```python
from build123d import *

# Parameters (mm, degrees)
JAW_BODY_DEPTH         = 64
PIVOT_BOSS_DEPTH       = 22
PIVOT_BORE_SKETCH_R    = 6
PIVOT_BORE_12_DEPTH    = 32
GUIDE_KEY_SKETCH_W     = 16
GUIDE_KEY_SKETCH_H     = 9
GUIDE_KEY_DEPTH        = 32
PIVOT_BOSS_FILLET_R3_R = 3
COUNTERBORE_SKETCH_R   = 5
COUNTERBORE_10X4_DEPTH = 4
SCREW_HOLE_SKETCH_R    = 3
SCREW_HOLE_6X4_DEPTH   = 4


with BuildPart() as part:
    # Jaw Body Profile Sketch → Jaw Body (new body)
    with BuildSketch(Plane.XY):
        Polygon((0, 0), (32, 0), (32, 10), (10, 10), (10, 36), (0, 36), align=None)
    extrude(amount=-JAW_BODY_DEPTH)

    # Pivot Boss Sketch → Pivot Boss (add)
    with BuildSketch(Plane(origin=(32, 0, 0), x_dir=(0, 0, -1), z_dir=(1, 0, 0))):
        with BuildLine():
            Line((4.5, 10), (16.574185034, 28.68413566))
            ThreePointArc((16.574185034, 28.68413566), (28.969550727, 35.965977968), (42.206819819, 30.358391585))
            Line((42.206819819, 30.358391585), (59.5, 10))
            Line((59.5, 10), (4.5, 10))
        make_face()
    extrude(amount=-PIVOT_BOSS_DEPTH)

    # Pivot Bore Sketch → Pivot Bore Ø12 (cut)
    with BuildSketch(Plane(origin=(32, 0, 0), x_dir=(0, 0, -1), z_dir=(1, 0, 0))):
        with Locations((30.01240619, 20)):
            Circle(PIVOT_BORE_SKETCH_R)
    extrude(amount=-PIVOT_BORE_12_DEPTH, mode=Mode.SUBTRACT)

    # Guide Key Sketch → Guide Key (add)
    with BuildSketch(Plane(origin=(32, 0, 0), x_dir=(0, 0, -1), z_dir=(1, 0, 0))):
        with Locations((32, -4.5)):
            Rectangle(GUIDE_KEY_SKETCH_W, GUIDE_KEY_SKETCH_H)
    extrude(amount=-GUIDE_KEY_DEPTH)

    # Pivot Boss Fillet R3
    pivot_boss_fillet_r3_edges = [part.edges().sort_by_distance(p)[0] for p in [
        (21, 10, -59.5),
        (21, 10, -4.5),
    ]]
    fillet(pivot_boss_fillet_r3_edges, radius=PIVOT_BOSS_FILLET_R3_R)

    # Counterbore Sketch → Counterbore Ø10x4 (cut)
    with BuildSketch(Plane(origin=(0, 36, 0), x_dir=(1, 0, 0), z_dir=(0, 1, 0))):
        with Locations(Location((20, 32, 0), (0, 0, 270))):
            Circle(COUNTERBORE_SKETCH_R)
    extrude(amount=-COUNTERBORE_10X4_DEPTH, mode=Mode.SUBTRACT)

    # Screw Hole Sketch → Screw Hole Ø6x4 (cut)
    with BuildSketch(Plane(origin=(0, 32, 0), x_dir=(1, 0, 0), z_dir=(0, 1, 0))):
        with Locations(Location((20, 32, 0), (0, 0, 270))):
            Circle(SCREW_HOLE_SKETCH_R)
    extrude(amount=-SCREW_HOLE_6X4_DEPTH, mode=Mode.SUBTRACT)


solid = part.part
```
CAD build for the part. Positions are in the model's coordinates, mm. A direction names the side the tool comes from. Round coordinates to 2 decimals unless told otherwise and drop trailing zeros. Loops run counter-clockwise (first coordinate to the right, second up) from the corner with the lowest first, then second, coordinate; pieces in that order, holes last. Notation, with made-up numbers: M -27.5,48.5 L 22.5,48.5 A19 cw 22.5,54.5 Z; hole C 82,60 d4. An arc over 180 degrees is marked long. Return JSON: item names as keys, results as strings. Group by question number.
(1) Saw through at B-B, the plane y = 20. List the corners of the cut face in (x, z).
(2) Saw through at C-C, the plane z = -32. List the corners of the cut face in (x, y), and give its area (3 significant figures).
(3) Drop flat-ended pins along their axis: P1, Ø9.5, axis at x = 20, z = -32, coming from the +Y side; P2, Ø7, axis at y = 20, z = -30.01, coming from the -X side; P3, Ø2, axis at x = 22.5, y = 19, coming from the -Z side; P4, Ø1.5, axis at x = 6.5, y = -4, coming from the +Z side. Give the stop position or say it passes through.
(4) Saw through at D-D, the plane y = -5. List the corners of the cut face in (x, z), and give its area (3 significant figures).
(5) Tool access for faces 4 (the flat face through (20, 28, -32)), 5 (the cylindrical face through (21.154, 35.353, -25.509)), 6 (the flat face through (21, 10, -62)), 7 (the flat face through (16, -5, -24)), 8 (the flat face through (16, 0, -52)): list every direction of +Z, -Z, +X, -X, +Y, -Y with a clear straight run to the whole face (end or side of a thin tool).
(6) Mould opens along Z. For faces 1 (the cylindrical face through (16.224, 17.702, -35.555)), 2 (the flat face through (32, 14, -32)), 3 (the cylindrical face through (20.846, 10.375, -4.32)) say: +Z half, -Z half, draft (parallel to the pull), parting line (faces both ways), or undercut.
(7) Wall check: probe 1 along X at (y, z) = (30.25, -32); probe 2 along Y at (x, z) = (9, -45); probe 3 along X at (y, z) = (26, -46). Give the ranges that are in metal, low to high. Write a range as [from, to].
(8) Saw through at A-A, the plane x = 29.5. List the corners of the cut face in (y, z), and give its area (3 significant figures).
Answer list:
{
 "1": {"outline": "M 0,-64 L 10,-64 L 10,-51.01 L 32,-51.01 L 32,-36.01 L 0,-36.01 Z; M 0,-24.01 L 32,-24.01 L 32,-10.96 L 10,-10.96 L 10,0 L 0,0 Z"},
 "2": {"outline": "M 0,-9 L 32,-9 L 32,14.34 L 0,14.34 Z; M 0,25.66 L 32,25.66 L 32,35.88 L 25,35.88 L 25,32 L 23,32 L 23,28 L 17,28 L 17,32 L 15,32 L 15,35.88 L 10,35.88 L 10,36 L 0,36 Z", "area": "1,010 mm2"},
 "3": {"P1": "y = 32", "P2": "through", "P3": "z = -52.7", "P4": "z = -24"},
 "4": {"outline": "M 0,-40 L 32,-40 L 32,-24 L 0,-24 Z", "area": "512 mm2"},
 "5": {"face 4": "+Y", "face 5": "+X, +Y", "face 6": "-Z, +X, +Y", "face 7": "+Z, +X, -X, -Y", "face 8": "-Z, +X, -X, -Y"},
 "6": {"face 1": "undercut", "face 2": "draft", "face 3": "+Z half"},
 "7": {"probe 1": "[0, 17], [23, 32]", "probe 2": "[0, 36]", "probe 3": "[0, 10]"},
 "8": {"outline": "M -9,-40 L 0,-40 L 0,-64 L 10,-64 L 10,-60.89 A3 cw 11.06,-58.6 L 30.36,-42.21 A16 ccw 28.68,-16.57 L 11.37,-5.39 A3 cw 10,-2.87 L 10,0 L 0,0 L 0,-24 L -9,-24 Z; hole C 20,-30.01 d12", "area": "1,580 mm2"}
}
